from build123d import *

# Parameters (mm, degrees)
SKETCH_1_R          = 18
EXTRUDE_519_DEPTH   = 31.9
SKETCH_2_OUTSIDE_W  = 363.728
SKETCH_2_OUTSIDE_H  = 355.584
SKETCH_2_OUTSIDE_R  = 26.322842148
CUT_EXTRUDE_1_DEPTH = 38
CUT_EXTRUDE_1_DRAFT = -75
SKETCH_3_OUTSIDE_W  = 363.728
SKETCH_3_OUTSIDE_H  = 355.584
SKETCH_3_OUTSIDE_R  = 26.322842148
CUT_EXTRUDE_2_DEPTH = 38
CUT_EXTRUDE_2_DRAFT = -75


with BuildPart() as part:
    # 草图1 → Extrude 519 (new body)
    with BuildSketch(Plane.XY):
        Polygon((15.1975, 26.322842148), (-15.1975, 26.322842148), (-30.395, 0), (-15.1975, -26.322842148), (15.1975, -26.322842148), (30.395, 0), align=None)
        Circle(SKETCH_1_R, mode=Mode.SUBTRACT)
    extrude(amount=EXTRUDE_519_DEPTH)


with BuildPart() as cut_extrude_1_tool:
    # 草图2 outside → 切除-拉伸1 (with draft: the straight prism first)
    with BuildSketch(Plane(origin=(0, 0, 0), x_dir=(-1, 0, 0), z_dir=(0, 0, -1))):
        Rectangle(SKETCH_2_OUTSIDE_W, SKETCH_2_OUTSIDE_H)
        Circle(SKETCH_2_OUTSIDE_R, mode=Mode.SUBTRACT)
    extrude(amount=-CUT_EXTRUDE_1_DEPTH)
    # 切除-拉伸1: the draft: its side faces are tilted about the plane it starts from
    cut_extrude_1_sides = [cut_extrude_1_tool.faces().sort_by_distance(p)[0] for p in [
        (0, -177.792, 19),
        (-181.864, 0, 19),
        (0, 177.792, 19),
        (181.864, 0, 19),
        (26.322842148, 0, 19),
    ]]
    draft(cut_extrude_1_sides, Plane(origin=(0, 0, 0), x_dir=(-1, 0, 0), z_dir=(0, 0, -1)), CUT_EXTRUDE_1_DRAFT)


with BuildPart() as part_1:
    add(part.part)

    # 切除-拉伸1: cut by cut_extrude_1_tool
    add(cut_extrude_1_tool.part, mode=Mode.SUBTRACT)


with BuildPart() as cut_extrude_2_tool:
    # 草图3 outside → 切除-拉伸2 (with draft: the straight prism first)
    with BuildSketch(Plane.XY.offset(31.9)):
        Rectangle(SKETCH_3_OUTSIDE_W, SKETCH_3_OUTSIDE_H)
        Circle(SKETCH_3_OUTSIDE_R, mode=Mode.SUBTRACT)
    extrude(amount=-CUT_EXTRUDE_2_DEPTH)
    # 切除-拉伸2: the draft: its side faces are tilted about the plane it starts from
    cut_extrude_2_sides = [cut_extrude_2_tool.faces().sort_by_distance(p)[0] for p in [
        (0, -177.792, 12.9),
        (181.864, 0, 12.9),
        (0, 177.792, 12.9),
        (-181.864, 0, 12.9),
        (-26.322842148, 0, 12.9),
    ]]
    draft(cut_extrude_2_sides, Plane.XY.offset(31.9), CUT_EXTRUDE_2_DRAFT)


with BuildPart() as part_2:
    add(part_1.part)

    # 切除-拉伸2: cut by cut_extrude_2_tool
    add(cut_extrude_2_tool.part, mode=Mode.SUBTRACT)


solid = part_2.part
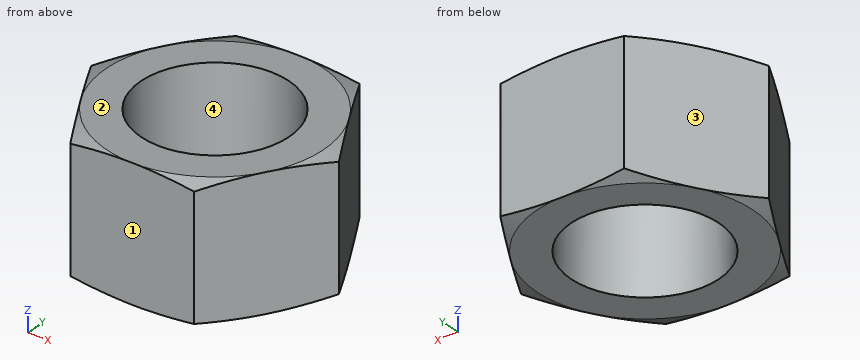
Check sheet for the modelled part. Datum: model origin and axes. Units: mm. Face numbers are marked on the shaded views. Round coordinates to 2 decimals unless told otherwise and drop trailing zeros. Loops run counter-clockwise (first coordinate to the right, second up) from the corner with the lowest first, then second, coordinate; pieces in that order, holes last. Notation, with made-up numbers: M 41.5,23 L 97.5,23 A18 cw 97.5,52 Z; hole C 35.25,67 d2. An arc over 180 degrees is marked long. One line per question, with ' | ' between items. Start each with the question number.
Item 1: Gauge pin test, flat ends, axial feed: pin 1 Ø8 at (x, y) = (7.5, 10.5) entering from +Z; pin 2 Ø1.5 at (y, z) = (17, 25.5) entering from +X; pin 3 Ø1.5 at (x, z) = (-22.5, 6) entering from -Y; pin 4 Ø6 at (y, z) = (-11, 16.5) entering from +X. Record the tip position at first contact, or that the pin passes through.
Item 2: Scan lines: probe 1 along Y at (x, z) = (14, 3); probe 2 along Y at (x, z) = (5, 8.5); probe 3 along X at (y, z) = (9.5, 23). Record each from-to range of solid material in increasing order.
Item 3: Release check for a two-part mould opening along Y. For the marked faces 1, 2, 3 and 4 record: released by +Y, released by -Y, zero draft, split by the parting line, or undercut.
Item 4: Section check A-A (z = 9). Record the boundary of the cut face in (x, y) (1 decimal).
Worked out:
1) pin 1: through | pin 2: x = 21.01 | pin 3: y = -14.97 | pin 4: x = 25.78
2) probe 1: -26.32 to -11.31, 11.31 to 26.32 | probe 2: -26.32 to -17.29, 17.29 to 26.32 | probe 3: -24.91 to -15.29, 15.29 to 24.91
3) face 1: released by -Y | face 2: zero draft | face 3: released by +Y | face 4: undercut
4) outline: M -30.4,0 L -15.2,-26.3 L 15.2,-26.3 L 30.4,0 L 15.2,26.3 L -15.2,26.3 Z; hole C 0,0 d36
